```python
from build123d import *

# Parameters (mm, degrees)
SKETCH_1_W      = 570
SKETCH_1_H      = 950
SKETCH_1_R      = 11
EXTRUDE_1_DEPTH = 30


with BuildPart() as part:
    # 草图1 → 凸台-拉伸1 (new body)
    with BuildSketch(Plane.XY):
        with Locations((1800, 1250)):
            Rectangle(SKETCH_1_W, SKETCH_1_H)
        with Locations((1580, 1665)):
            Circle(SKETCH_1_R, mode=Mode.SUBTRACT)
        with Locations((1710, 1665)):
            Circle(SKETCH_1_R, mode=Mode.SUBTRACT)
        with Locations((1890, 1665)):
            Circle(SKETCH_1_R, mode=Mode.SUBTRACT)
        with Locations((2020, 1665)):
            Circle(SKETCH_1_R, mode=Mode.SUBTRACT)
        with Locations((1710, 1372.5)):
            Circle(SKETCH_1_R, mode=Mode.SUBTRACT)
        with Locations((1890, 1372.5)):
            Circle(SKETCH_1_R, mode=Mode.SUBTRACT)
        with Locations(Location((1710, 1127.5, 0), (0, 0, 180))):
            Circle(SKETCH_1_R, mode=Mode.SUBTRACT)
        with Locations(Location((1890, 1127.5, 0), (0, 0, 180))):
            Circle(SKETCH_1_R, mode=Mode.SUBTRACT)
        with Locations(Location((2020, 835, 0), (0, 0, 180))):
            Circle(SKETCH_1_R, mode=Mode.SUBTRACT)
        with Locations(Location((1890, 835, 0), (0, 0, 180))):
            Circle(SKETCH_1_R, mode=Mode.SUBTRACT)
        with Locations(Location((1710, 835, 0), (0, 0, 180))):
            Circle(SKETCH_1_R, mode=Mode.SUBTRACT)
        with Locations(Location((1580, 835, 0), (0, 0, 180))):
            Circle(SKETCH_1_R, mode=Mode.SUBTRACT)
        with BuildLine():
            Line((1840, 1025), (1760, 1025))
            ThreePointArc((1760, 1025), (1752.928932188, 1027.928932188), (1750, 1035))
            Line((1750, 1035), (1750, 1465))
            ThreePointArc((1750, 1465), (1752.928932188, 1472.071067812), (1760, 1475))
            Line((1760, 1475), (1840, 1475))
            ThreePointArc((1840, 1475), (1847.071067812, 1472.071067812), (1850, 1465))
            Line((1850, 1465), (1850, 1035))
            ThreePointArc((1850, 1035), (1847.071067812, 1027.928932188), (1840, 1025))
        make_face(mode=Mode.SUBTRACT)
        with BuildLine():
            Line((1655, 1510), (1655, 1310))
            ThreePointArc((1655, 1310), (1625, 1280), (1595, 1310))
            Line((1595, 1310), (1595, 1510))
            ThreePointArc((1595, 1510), (1625, 1540), (1655, 1510))
        make_face(mode=Mode.SUBTRACT)
        with BuildLine():
            Line((2005, 1510), (2005, 1310))
            ThreePointArc((2005, 1310), (1975, 1280), (1945, 1310))
            Line((1945, 1310), (1945, 1510))
            ThreePointArc((1945, 1510), (1975, 1540), (2005, 1510))
        make_face(mode=Mode.SUBTRACT)
        with BuildLine():
            Line((2005, 990), (2005, 1190))
            ThreePointArc((2005, 1190), (1975, 1220), (1945, 1190))
            Line((1945, 1190), (1945, 990))
            ThreePointArc((1945, 990), (1975, 960), (2005, 990))
        make_face(mode=Mode.SUBTRACT)
        with BuildLine():
            Line((1655, 990), (1655, 1190))
            ThreePointArc((1655, 1190), (1625, 1220), (1595, 1190))
            Line((1595, 1190), (1595, 990))
            ThreePointArc((1595, 990), (1625, 960), (1655, 990))
        make_face(mode=Mode.SUBTRACT)
    extrude(amount=EXTRUDE_1_DEPTH)


solid = part.part
```
Build history of the part. All positions in model axes, mm. A direction names the side the tool comes from. Coordinates: 2 decimals unless noted, no trailing zeros. Order: outer loops, then holes, each group sorted by start corner. A loop starts at its lowest first (then second) coordinate and runs counter-clockwise, first axis right, second up. Notation, with made-up numbers: (24.25, -23) -> (73.25, -23) arc R32 ccw to (73.25, 11) -> close; hole circle Ø10 at (-32.5, 46). An arc over 180 degrees is marked (long way). Answer in a Markdown table with one row per item. Add a question column.
Q1. Band-saw the part on B-B, the plane y = 1150.5. List the corners of the cut face in (x, z), then the cut area to 3 significant figures.
Q2. Wall check: line 1 along Y through (x, z) = (1710, 20.25); line 2 along X through (y, z) = (1665, 7.75); line 3 along X through (y, z) = (1126.5, 25.75). Give the ranges that are in metal, low to high. Write a range as [from, to].
Q3. Band-saw the part on D-D, the plane y = 1665. List the corners of the cut face in (x, z), then the cut area to 3 significant figures.
Q4. Drop a flat-ended pin along its axis: pin 1 (6 mm diameter, centred on x = 1978, y = 1538.5, fed in from +Z). Give the stop position or say it passes through.
Q5. Which spindle directions (+Z, -Z, +X, -X, +Y, -Y) get a long thin tool onto all of the face, cutting with end or side? Do faces 1 (the face through (1975.66, 1219.993, 14.79)), 2 (the face through (1859, 1257, 30)). Say none if no direction does.
Q6. Band-saw the part on C-C, the plane x = 1975. List the corners of the cut face in (y, z), then the cut area to 3 significant figures.
Q7. Band-saw the part on A-A, the plane x = 1710. List the corners of the cut face in (y, z).
Q8. Mould opens along Y. For faces 3 (the face through (1796, 775, 15)), 4 (the face through (1879.839, 839.213, 14.79)), 5 (the face through (1859, 1257, 0)) say: +Y half, -Y half, draft (parallel to the pull), parting line (faces both ways), or undercut.
Answers follow:
| question | item | result |
|---|---|---|
| 1 | outline | (1515, 0) -> (1595, 0) -> (1595, 30) -> (1515, 30) -> close; (1655, 0) -> (1750, 0) -> (1750, 30) -> (1655, 30) -> close; (1850, 0) -> (1945, 0) -> (1945, 30) -> (1850, 30) -> close; (2005, 0) -> (2085, 0) -> (2085, 30) -> (2005, 30) -> close |
| 1 | area | 10,500 mm^2 |
| 2 | line 1 | [775, 824], [846, 1116.5], [1138.5, 1361.5], [1383.5, 1654], [1676, 1725] |
| 2 | line 2 | [1515, 1569], [1591, 1699], [1721, 1879], [1901, 2009], [2031, 2085] |
| 2 | line 3 | [1515, 1595], [1655, 1699.05], [1720.95, 1750], [1850, 1879.05], [1900.95, 1945], [2005, 2085] |
| 3 | outline | (1515, 0) -> (1569, 0) -> (1569, 30) -> (1515, 30) -> close; (1591, 0) -> (1699, 0) -> (1699, 30) -> (1591, 30) -> close; (1721, 0) -> (1879, 0) -> (1879, 30) -> (1721, 30) -> close; (1901, 0) -> (2009, 0) -> (2009, 30) -> (1901, 30) -> close; (2031, 0) -> (2085, 0) -> (2085, 30) -> (2031, 30) -> close |
| 3 | area | 14,500 mm^2 |
| 4 | pin 1 | z = 30 |
| 5 | face 1 | +Z, -Z |
| 5 | face 2 | +Z, +X, -X, +Y, -Y |
| 6 | outline | (775, 0) -> (960, 0) -> (960, 30) -> (775, 30) -> close; (1220, 0) -> (1280, 0) -> (1280, 30) -> (1220, 30) -> close; (1540, 0) -> (1725, 0) -> (1725, 30) -> (1540, 30) -> close |
| 6 | area | 12,900 mm^2 |
| 7 | outline | (775, 0) -> (824, 0) -> (824, 30) -> (775, 30) -> close; (846, 0) -> (1116.5, 0) -> (1116.5, 30) -> (846, 30) -> close; (1138.5, 0) -> (1361.5, 0) -> (1361.5, 30) -> (1138.5, 30) -> close; (1383.5, 0) -> (1654, 0) -> (1654, 30) -> (1383.5, 30) -> close; (1676, 0) -> (1725, 0) -> (1725, 30) -> (1676, 30) -> close |
| 8 | face 3 | -Y half |
| 8 | face 4 | undercut |
| 8 | face 5 | draft |
